Verification items for the finished model (mm, model axes). Face numbers are marked on the shaded views. A direction names the side the tool comes from. Give positions to 0.01 mm unless a question says otherwise; leave off trailing zeros. Loops run counter-clockwise (first coordinate to the right, second up) from the corner with the lowest first, then second, coordinate; pieces in that order, holes last. Notation, with made-up numbers: (57.25, -24.5) - (86.25, -24.5) arc R27 cw to (86.25, 3.5) - close; hole circle Ø4 at (-40, 24). An arc over 180 degrees is marked (long way). One line per item, written item: value. Start each with the question number.
1. Sectioned sample at C-C (z = -80). Record the cut outline in (x, y), plus the area to 3 significant figures.
2. Access from +Z, -Z, +X, -X, +Y, -Y to the whole of each face (thin tool, end or side, straight path). Record for the marked faces 5, 6 and 7.
3. Sectioned sample at A-A (y = 45). Record the cut outline in (x, z), plus the area to 3 significant figures.
4. Gauge pin test, flat ends, axial feed: pin 1 (3 mm diameter, centred on x = 79.5, y = 58, fed in from +Z); pin 2 (8 mm diameter, centred on y = 16.5, z = -35, fed in from +X); pin 3 (1.5 mm diameter, centred on x = 53.5, z = 31.5, fed in from +Y); pin 4 (6 mm diameter, centred on y = 21.5, z = -71, fed in from -X). Record the tip position at first contact, or that the pin passes through.
5. Scan lines: L1, parallel to Z at x = 64.5, y = 78.5; L2, parallel to Y at x = 24, z = -18; L3, parallel to Z at x = 62, y = 21. Record each from-to range of solid material in increasing order. Write a range as [from, to].
6. Sectioned sample at D-D (y = 60). Record the cut outline in (x, z).
7. Sectioned sample at B-B (z = -5). Record the cut outline in (x, y).
8. Mould release check, pull along Z, two halves, no side actions. Record for the marked faces 1, 2, 3 and 4: pulls with the +Z half, pulls with the -Z half, needs draft (parallel to the pull), parting line crosses it, or undercut.
from build123d import *

# Parameters (mm, degrees)
SKETCH_1_W          = 90
SKETCH_1_H          = 90
EXTRUDE_1_DEPTH     = 10
SKETCH_2_R          = 35
EXTRUDE_2_DEPTH     = 3
SKETCH_3_R          = 17.5
EXTRUDE_3_DEPTH     = 0.5
EXTRUDE_4_DEPTH     = 36.5
CUT_EXTRUDE_1_REACH = 135.417
SKETCH_5_R          = 3.25
SKETCH_7_W          = 90
SKETCH_7_H          = 90
EXTRUDE_5_DEPTH     = 91
SKETCH_8_R          = 20
CUT_EXTRUDE_2_DEPTH = 48
FILLET_1_R          = 5
SKETCH_6_OUTSIDE_W  = 129.99
SKETCH_6_OUTSIDE_H  = 129.99
SKETCH_6_OUTSIDE_R  = 58
CUT_EXTRUDE_3_DEPTH = 163.483845351


with BuildPart() as part:
    # 草图1 → 拉伸1 (new body)
    with BuildSketch(Plane.XY):
        with Locations((45, 45)):
            Rectangle(SKETCH_1_W, SKETCH_1_H)
    extrude(amount=EXTRUDE_1_DEPTH)

    # 草图2 → 拉伸2 (add)
    with BuildSketch(Plane.XY.offset(10)):
        with Locations(Location((45, 45, 0), (0, 0, 180))):
            Circle(SKETCH_2_R)
    extrude(amount=EXTRUDE_2_DEPTH)

    # 草图3 → 拉伸3 (add)
    with BuildSketch(Plane.XY.offset(13)):
        with Locations((45, 45)):
            Circle(SKETCH_3_R)
    extrude(amount=EXTRUDE_3_DEPTH)

    # 草图4 → 拉伸4 (add)
    with BuildSketch(Plane.XY.offset(13.5)):
        with BuildLine():
            Line((38.291796068, 51), (51.708203932, 51))
            ThreePointArc((51.708203932, 51), (45, 36), (38.291796068, 51))
        make_face()
    extrude(amount=EXTRUDE_4_DEPTH)

    # 草图5 → 切除-拉伸1 (cut, up to next)
    with BuildSketch(Plane.XY.offset(10), mode=Mode.PRIVATE) as cut_extrude_1_sk1:
        with Locations((9.644660941, 80.355339059)):
            Circle(SKETCH_5_R)
    cut_extrude_1_tool1 = extrude(cut_extrude_1_sk1.sketch, amount=-CUT_EXTRUDE_1_REACH, mode=Mode.PRIVATE) & part.part
    # 草图5 → 切除-拉伸1 (cut, up to next)
    with BuildSketch(Plane.XY.offset(10), mode=Mode.PRIVATE) as cut_extrude_1_sk2:
        with Locations(Location((80.355339059, 80.355339059, 0), (0, 0, 180))):
            Circle(SKETCH_5_R)
    cut_extrude_1_tool2 = extrude(cut_extrude_1_sk2.sketch, amount=-CUT_EXTRUDE_1_REACH, mode=Mode.PRIVATE) & part.part
    # 草图5 → 切除-拉伸1 (cut, up to next)
    with BuildSketch(Plane.XY.offset(10), mode=Mode.PRIVATE) as cut_extrude_1_sk3:
        with Locations((80.355339059, 9.644660941)):
            Circle(SKETCH_5_R)
    cut_extrude_1_tool3 = extrude(cut_extrude_1_sk3.sketch, amount=-CUT_EXTRUDE_1_REACH, mode=Mode.PRIVATE) & part.part
    # 草图5 → 切除-拉伸1 (cut, up to next)
    with BuildSketch(Plane.XY.offset(10), mode=Mode.PRIVATE) as cut_extrude_1_sk4:
        with Locations(Location((9.644660941, 9.644660941, 0), (0, 0, 180))):
            Circle(SKETCH_5_R)
    cut_extrude_1_tool4 = extrude(cut_extrude_1_sk4.sketch, amount=-CUT_EXTRUDE_1_REACH, mode=Mode.PRIVATE) & part.part
    add(cut_extrude_1_tool1.solids().sort_by_distance((9.644661, 80.355339, 10))[0], mode=Mode.SUBTRACT)
    add(cut_extrude_1_tool2.solids().sort_by_distance((80.355339, 80.355339, 10))[0], mode=Mode.SUBTRACT)
    add(cut_extrude_1_tool3.solids().sort_by_distance((80.355339, 9.644661, 10))[0], mode=Mode.SUBTRACT)
    add(cut_extrude_1_tool4.solids().sort_by_distance((9.644661, 9.644661, 10))[0], mode=Mode.SUBTRACT)

    # 草图7 → 拉伸5 (add)
    with BuildSketch(Plane(origin=(0, 0, 0), x_dir=(-1, 0, 0), z_dir=(0, 0, -1))):
        with Locations((-45, 45)):
            Rectangle(SKETCH_7_W, SKETCH_7_H)
    extrude(amount=EXTRUDE_5_DEPTH)

    # 草图8 → 切除-拉伸2 (cut)
    with BuildSketch(Plane.XY):
        with Locations((90, 90)):
            Circle(SKETCH_8_R)
        with Locations((90, 0)):
            Circle(SKETCH_8_R)
        Circle(SKETCH_8_R)
        with Locations((0, 90)):
            Circle(SKETCH_8_R)
    extrude(amount=-CUT_EXTRUDE_2_DEPTH, mode=Mode.SUBTRACT)

    # 圆角1
    fillet_1_edges = [part.edges().sort_by_distance(p)[0] for p in [
        (70, 90, -24),
        (90, 70, -24),
        (70, 0, -24),
        (90, 20, -24),
        (20, 0, -24),
        (0, 20, -24),
        (20, 90, -24),
        (0, 70, -24),
    ]]
    fillet(fillet_1_edges, radius=FILLET_1_R)

    # 草图6 outside → 切除-拉伸3 (cut, through all)
    with BuildSketch(Plane.XY.offset(10)):
        with Locations((45, 45)):
            Rectangle(SKETCH_6_OUTSIDE_W, SKETCH_6_OUTSIDE_H)
        with Locations((45, 45)):
            Circle(SKETCH_6_OUTSIDE_R, mode=Mode.SUBTRACT)
    extrude(amount=-CUT_EXTRUDE_3_DEPTH, mode=Mode.SUBTRACT)


solid = part.part
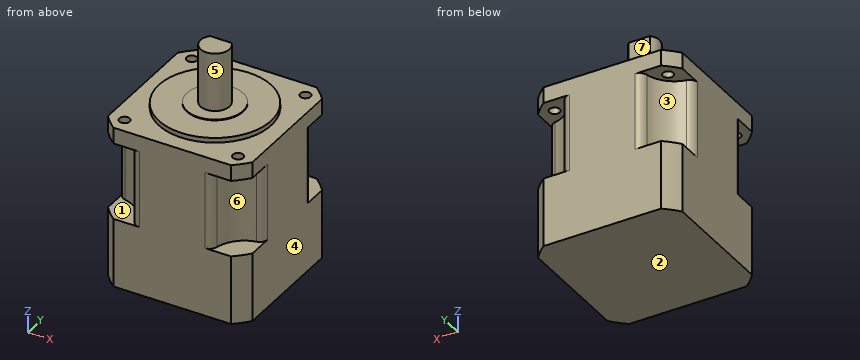
Results are:
1. outline: (0, 8.41) arc R58 ccw to (8.41, 0) - (81.59, 0) arc R58 ccw to (90, 8.41) - (90, 81.59) arc R58 ccw to (81.59, 90) - (8.41, 90) arc R58 ccw to (0, 81.59) - close
1. area: 7,970 mm^2
2. face 5: +Z
2. face 6: +X, -Y
2. face 7: +Z, +X, -X, +Y
3. outline: (0, -91) - (90, -91) - (90, 10) - (80, 10) - (80, 13) - (62.5, 13) - (62.5, 13.5) - (54, 13.5) - (54, 50) - (36, 50) - (36, 13.5) - (27.5, 13.5) - (27.5, 13) - (10, 13) - (10, 10) - (0, 10) - close
3. area: 9,970 mm^2
4. pin 1: stops at z = 10
4. pin 2: stops at x = 88.01
4. pin 3: stops at y = 49.58
4. pin 4: stops at x = 0
5. L1: z = [-91, 10]
5. L2: y = [0.02, 89.98]
5. L3: z = [-91, 13]
6. outline: (0, -91) - (90, -91) - (90, 10) - (76.62, 10) - (76.62, 13) - (54.01, 13) - (54.01, 13.5) - (35.99, 13.5) - (35.99, 13) - (13.38, 13) - (13.38, 10) - (0, 10) - close
7. outline: (0, 24.49) arc R5 ccw to (4, 19.6) arc R20 cw to (19.6, 4) arc R5 ccw to (24.49, 0) - (65.51, 0) arc R5 ccw to (70.4, 4) arc R20 cw to (86, 19.6) arc R5 ccw to (90, 24.49) - (90, 65.51) arc R5 ccw to (86, 70.4) arc R20 cw to (70.4, 86) arc R5 ccw to (65.51, 90) - (24.49, 90) arc R5 ccw to (19.6, 86) arc R20 cw to (4, 70.4) arc R5 ccw to (0, 65.51) - close
8. face 1: undercut
8. face 2: pulls with the -Z half
8. face 3: undercut
8. face 4: needs draft
